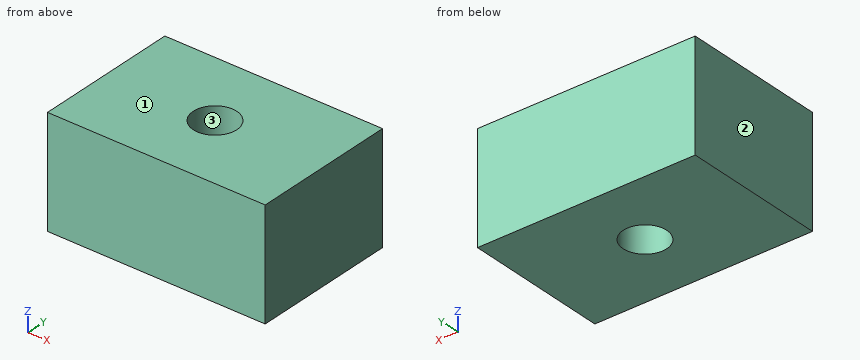
```python
from build123d import *

# Parameters (mm, degrees)
SKETCH1_W               = 30
SKETCH1_H               = 20
BOSS_EXTRUDE1_DEPTH     = 15
CUT_EXTRUDE1_DEPTH      = 24.452078799
CUT_EXTRUDE1_DEPTH_BACK = 24.452078799
SKETCH2_R               = 3


with BuildPart() as part:
    # Sketch1 → Boss-Extrude1 (new body)
    with BuildSketch(Plane.XY):
        Rectangle(SKETCH1_W, SKETCH1_H)
    extrude(amount=BOSS_EXTRUDE1_DEPTH)

    # Sketch2 → Cut-Extrude1 (cut, two sides: drawn at the far end of the back side and taken through both)
    with BuildSketch(Plane.XY.offset(15).offset(-CUT_EXTRUDE1_DEPTH_BACK)):
        Circle(SKETCH2_R)
    extrude(amount=CUT_EXTRUDE1_DEPTH + CUT_EXTRUDE1_DEPTH_BACK, mode=Mode.SUBTRACT)


solid = part.part
```
Design review of the part built by this model. Coordinates are the model's own, in mm. Face numbers are marked on the shaded views. Coordinates: 2 decimals unless noted, no trailing zeros. Order: outer loops, then holes, each group sorted by start corner. A loop starts at its lowest first (then second) coordinate and runs counter-clockwise, first axis right, second up. Notation, with made-up numbers: (61.25, 14) - (81.25, 14) arc R21 ccw to (81.25, 26) - close; hole circle Ø4 at (4.5, 83.5). An arc over 180 degrees is marked (long way). One line per question, with ' | ' between items.
Q1. Consider section C-C, the plane z = 4. Give the boundary of the cut face in (x, y).
Answer key:
outline: (-15, -10) - (15, -10) - (15, 10) - (-15, 10) - close; hole circle Ø6 at (0, 0)
Q2. Consider section A-A, the plane x = 0. Give the boundary of the cut face in (y, z), then the cut area to 3 significant figures.
Answer key:
outline: (-10, 0) - (-3, 0) - (-3, 15) - (-10, 15) - close; (3, 0) - (10, 0) - (10, 15) - (3, 15) - close | area: 210 mm2
Q3. Clearance check with flat-ended pins moving along their axes: pin 1 Ø3.5 at (x, y) = (0, 0) entering from +Z; pin 2 Ø2 at (x, y) = (-9.5, -0.5) entering from -Z. State where each tip first meets the part, or that it passes through.
Answer key:
pin 1: passes through | pin 2: stops at z = 0
Q4. Consider section B-B, the plane y = 0. Give the boundary of the cut face in (x, z).
Answer key:
outline: (-15, 0) - (-3, 0) - (-3, 15) - (-15, 15) - close; (3, 0) - (15, 0) - (15, 15) - (3, 15) - close
Q5. To check wall thickness, follow line 1 along X through (y, z) = (0, 8); line 2 along Y through (x, z) = (0, 4); line 3 along Y through (x, z) = (-2.5, 11). State the ranges of each line that lie inside material, in increasing order.
Answer key:
line 1: x = -15 to -3, 3 to 15 | line 2: y = -10 to -3, 3 to 10 | line 3: y = -10 to -1.66, 1.66 to 10
Q6. The part is to be moulded in two halves that separate along X. For the marked faces 1, 2 and 3, say which applies: +X half, -X half, draft (parallel to the pull), parting line (faces both ways), or undercut.
Answer key:
face 1: draft | face 2: -X half | face 3: undercut
